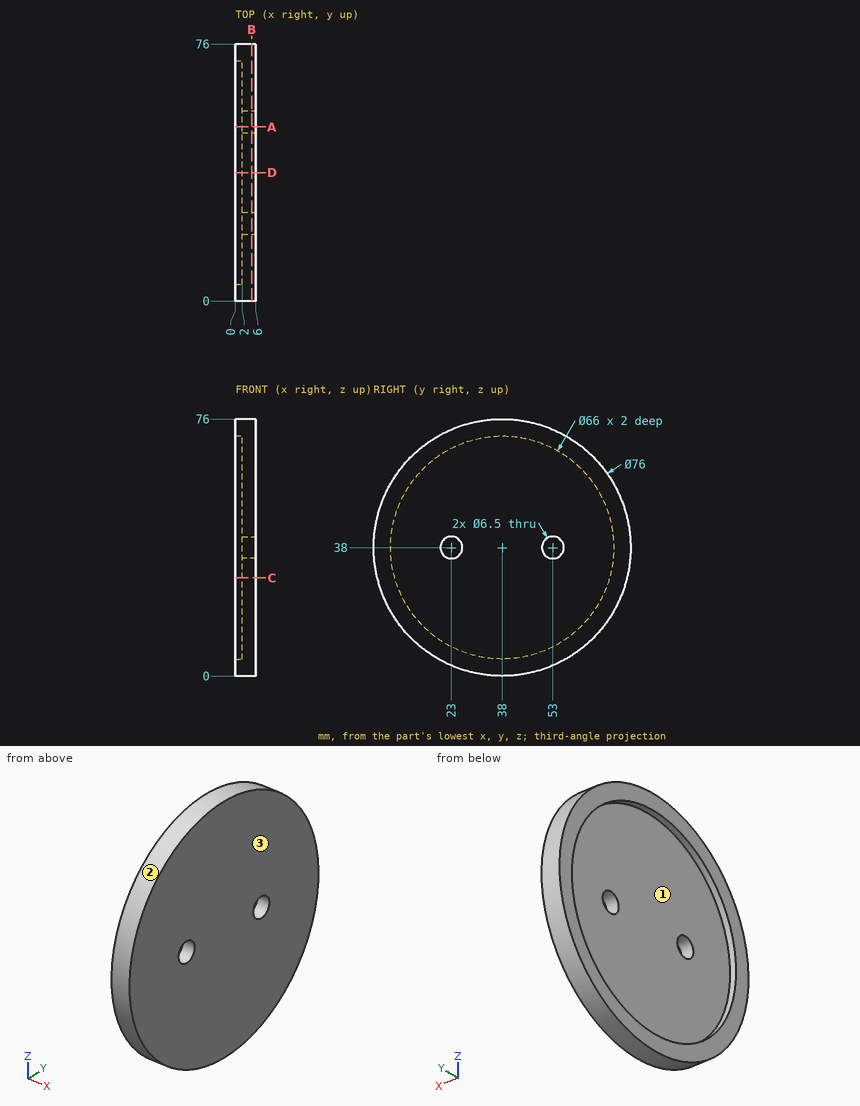
Check sheet for the drawn part. Datum: minimum x, y, z corner. Units: mm. Round coordinates to 2 decimals unless told otherwise and drop trailing zeros. Loops run counter-clockwise (first coordinate to the right, second up) from the corner with the lowest first, then second, coordinate; pieces in that order, holes last. Notation, with made-up numbers: (-13, 11) -> (26, 11) arc R9 cw to (26, 20) -> close; hole circle Ø9 at (-34, 83.5). An arc over 180 degrees is marked (long way). Put each result on its own line as item: value. Start each with the question number.
1. Section check A-A (y = 51.5). Enter the section's corners in (x, z), plus the area to 3 significant figures.
2. Draft check along Y on the marked faces 1, 2 and 3. Enter one of: +Y half, -Y half, draft (parallel to the pull), parting line (faces both ways), or undercut.
3. Gauge pin test, flat ends, axial feed: pin 1 (3 mm diameter, centred on x = 2.5, z = 41, fed in from +Y); pin 2 (2 mm diameter, centred on y = 11.5, z = 67, fed in from +X); pin 3 (6 mm diameter, centred on y = 50, z = 61, fed in from -X); pin 4 (7.5 mm diameter, centred on y = 53, z = 38, fed in from +X). Record the tip position at first contact, or that the pin passes through.
4. Section check C-C (z = 29). Enter the section's corners in (x, y), plus the area to 3 significant figures.
5. Section check B-B (x = 4.8). Enter the section's corners in (y, z).
6. Section check D-D (y = 38). Enter the section's corners in (x, z).
7. Scan lines: probe 1 along Y at (x, z) = (4.9, 38); probe 2 along X at (y, z) = (47.5, 26); probe 3 along Y at (x, z) = (0.8, 67). Record each from-to range of solid material in increasing order.
Findings:
1. outline: (0, 2.48) -> (6, 2.48) -> (6, 35.12) -> (2, 35.12) -> (2, 7.89) -> (0, 7.89) -> close; (0, 68.11) -> (2, 68.11) -> (2, 40.88) -> (6, 40.88) -> (6, 73.52) -> (0, 73.52) -> close
1. area: 283 mm^2
2. face 1: undercut
2. face 2: parting line
2. face 3: draft
3. pin 1: stops at y = 75.97
3. pin 2: passes through
3. pin 3: stops at x = 2
3. pin 4: stops at x = 6
4. outline: (0, 1.08) -> (6, 1.08) -> (6, 74.92) -> (0, 74.92) -> (0, 69.75) -> (2, 69.75) -> (2, 6.25) -> (0, 6.25) -> close
4. area: 316 mm^2
5. outline: circle Ø76 at (38, 38); hole circle Ø6.5 at (23, 38); hole circle Ø6.5 at (53, 38)
6. outline: (0, 0) -> (6, 0) -> (6, 76) -> (0, 76) -> (0, 71) -> (2, 71) -> (2, 5) -> (0, 5) -> close
7. probe 1: y = 0 to 19.75, 26.25 to 49.75, 56.25 to 76
7. probe 2: x = 2 to 6
7. probe 3: y = 13.44 to 22.25, 53.75 to 62.56
